```python
from build123d import *

# Parameters (mm, degrees)
SKETCH1_R               = 7.5
BOSS_EXTRUDE1_DEPTH     = 30
SKETCH2_R               = 45
SKETCH2_R_2             = 40
EXTRUDE_THIN1_DEPTH     = 30
SKETCH5_W               = 4
SKETCH5_H               = 36.329230713
EXTRUDE_THIN3_DEPTH     = 30
CIRPATTERN4_COUNT       = 6
CUT_EXTRUDE1_DEPTH      = 124.778996688
CUT_EXTRUDE1_DEPTH_BACK = 124.778996688
SKETCH6_R               = 4


with BuildPart() as part:
    # Sketch1 → Boss-Extrude1 (new body)
    with BuildSketch(Plane.XY):
        with Locations((10, -61.753173354)):
            Circle(SKETCH1_R)
    extrude(amount=BOSS_EXTRUDE1_DEPTH)



with BuildPart() as body_2:
    # Sketch2 → Extrude-Thin1 (new body)
    with BuildSketch(Plane.XY.offset(30)):
        with Locations((10, -61.753173354)):
            Circle(SKETCH2_R)
        with Locations((10, -61.753173354)):
            Circle(SKETCH2_R_2, mode=Mode.SUBTRACT)
    extrude(amount=-EXTRUDE_THIN1_DEPTH)


with BuildPart() as part_1:
    add(part.part)

    add(body_2.part)  # Extrude-Thin3 merges body 2
    # Sketch5 → Extrude-Thin3 (add)
    with BuildSketch(Plane.XY.offset(30)):
        with Locations((10, -39.294001794)):
            Rectangle(SKETCH5_W, SKETCH5_H)
    extrude_thin3 = extrude(amount=-EXTRUDE_THIN3_DEPTH)

    # CirPattern4: Extrude-Thin3 ×6 about axis
    cirpattern4_axis = Axis((10, -61.753173354, 0), (0, 0, 1))
    for i in range(1, CIRPATTERN4_COUNT):
        add(extrude_thin3.rotate(cirpattern4_axis, i * 360 / CIRPATTERN4_COUNT))

    # Sketch6 → Cut-Extrude1 (cut, two sides: drawn at the far end of the back side and taken through both)
    with BuildSketch(Plane.XY.offset(30).offset(-CUT_EXTRUDE1_DEPTH_BACK)):
        with Locations((10, -61.753173354)):
            Circle(SKETCH6_R)
    extrude(amount=CUT_EXTRUDE1_DEPTH + CUT_EXTRUDE1_DEPTH_BACK, mode=Mode.SUBTRACT)


solid = part_1.part
```
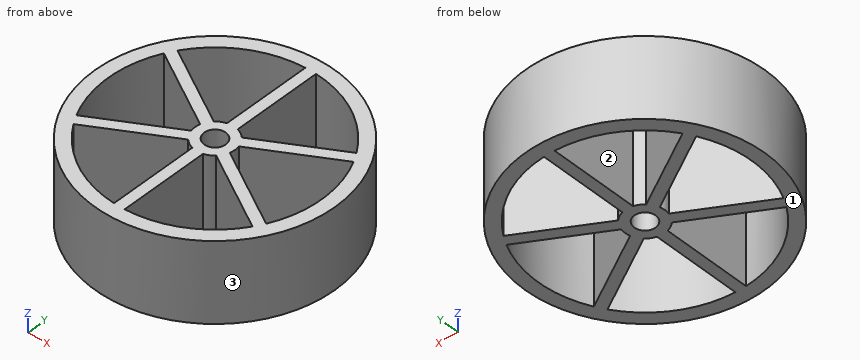
Geometry: final body of the model. Coordinates: model frame, mm. Face numbers are marked on the shaded views. Coordinates: 2 decimals unless noted, no trailing zeros. Order: outer loops, then holes, each group sorted by start corner. A loop starts at its lowest first (then second) coordinate and runs counter-clockwise, first axis right, second up.
Item 1: Material intervals for line 1 along Y through (x, z) = (10, 8.5); line 2 along X through (y, z) = (-94, 18.5); line 3 along X through (y, z) = (-34, 7.25), sorted ascending.
Answer:
line 1: y = -106.75 to -65.75, -57.75 to -16.75
line 2: x = -21.39 to -13.67, 8 to 12, 33.67 to 41.39
line 3: x = -25.42 to -18.81, 8 to 12, 38.81 to 45.42
Item 2: Contact query for flat-ended pins moving along their axis: P1, Ø2, axis at x = 24.5, z = 14.5, coming from the +Y side; P2, Ø5, axis at y = -41, z = 16.5, coming from the +X side; P3, Ø1.5, axis at x = 24.5, z = 19.5, coming from the +Y side; P4, Ø13, axis at x = 10, y = -61.75, coming from the -Z side. Output: stop coordinate, or through.
Answer:
P1: stops at y = -18.83
P2: stops at x = 51.13
P3: stops at y = -18.91
P4: stops at z = 0
Item 3: Section query D-D (x = -3.5). Output: boundary loops of the cut face in (y, z).
Answer:
outline: (-104.68, 0) - (-99.41, 0) - (-99.41, 30) - (-104.68, 30) - close; (-71.86, 0) - (-67.24, 0) - (-67.24, 30) - (-71.86, 30) - close; (-56.27, 0) - (-51.65, 0) - (-51.65, 30) - (-56.27, 30) - close; (-24.1, 0) - (-18.83, 0) - (-18.83, 30) - (-24.1, 30) - close
Item 4: Section query A-A (x = 10). Output: boundary loops of the cut face in (y, z).
Answer:
outline: (-106.75, 0) - (-65.75, 0) - (-65.75, 30) - (-106.75, 30) - close; (-57.75, 0) - (-16.75, 0) - (-16.75, 30) - (-57.75, 30) - close
Item 5: Draft query along X for the marked faces 1, 2 and 3. Return one class per face: released by +X, released by -X, zero draft, split by the parting line, or undercut.
Answer:
face 1: zero draft
face 2: undercut
face 3: split by the parting line
Item 6: Section query B-B (y = -96). Output: boundary loops of the cut face in (x, z).
Answer:
outline: (-19.19, 0) - (-10.67, 0) - (-10.67, 30) - (-19.19, 30) - close; (8, 0) - (12, 0) - (12, 30) - (8, 30) - close; (30.67, 0) - (39.19, 0) - (39.19, 30) - (30.67, 30) - close
Item 7: Section query C-C (z = 17). Output: boundary loops of the cut face in (x, y), then the cut area to 3 significant figures.
Answer:
outline: circle Ø90 at (10, -61.75); hole (-25.6, -80) - (2.74, -63.64) arc R7.5 cw to (2.74, -59.87) - (-25.6, -43.51) arc R40 ccw to start; hole (-23.6, -83.46) arc R40 ccw to (8, -101.7) - (8, -68.98) arc R7.5 cw to (4.74, -67.1) - close; hole (-23.6, -40.05) - (4.74, -56.41) arc R7.5 cw to (8, -54.52) - (8, -21.8) arc R40 ccw to start; hole circle Ø8 at (10, -61.75); hole (12, -101.7) arc R40 ccw to (43.6, -83.46) - (15.26, -67.1) arc R7.5 cw to (12, -68.98) - close; hole (12, -54.52) arc R7.5 cw to (15.26, -56.41) - (43.6, -40.05) arc R40 ccw to (12, -21.8) - close; hole (17.26, -63.64) - (45.6, -80) arc R40 ccw to (45.6, -43.51) - (17.26, -59.87) arc R7.5 cw to start
area: 2,240 mm2
